from build123d import *

# Parameters (mm, degrees)
SKETCH1_R           = 5
BOSS_EXTRUDE1_DEPTH = 6
SKETCH2_R           = 3
BOSS_EXTRUDE2_DEPTH = 25
CHAMFER1_SIZE       = 0.3
CUT_EXTRUDE1_DEPTH  = 3


with BuildPart() as part:
    # Sketch1 → Boss-Extrude1 (new body)
    with BuildSketch(Plane.XY):
        Circle(SKETCH1_R)
    extrude(amount=BOSS_EXTRUDE1_DEPTH)

    # Sketch2 → Boss-Extrude2 (add)
    with BuildSketch(Plane.XY.offset(6)):
        Circle(SKETCH2_R)
    extrude(amount=BOSS_EXTRUDE2_DEPTH)

    # Chamfer1
    chamfer1_edges = [part.edges().sort_by_distance(p)[0] for p in [
        (-5, 0, 0),
        (-5, 0, 6),
    ]]
    chamfer(chamfer1_edges, length=CHAMFER1_SIZE)

    # Sketch3 → Cut-Extrude1 (cut)
    with BuildSketch(Plane(origin=(0, 0, 0), x_dir=(-1, 0, 0), z_dir=(0, 0, -1))):
        Polygon((0, 2.42932406), (-2.10385635, 1.21466203), (-2.10385635, -1.21466203), (0, -2.42932406), (2.10385635, -1.21466203), (2.10385635, 1.21466203), align=None)
    extrude(amount=-CUT_EXTRUDE1_DEPTH, mode=Mode.SUBTRACT)


solid = part.part
Can you work these out from the model? Positions are in its coordinate system, mm. A direction names the side the tool comes from. Give positions to 0.01 mm unless a question says otherwise; leave off trailing zeros. Write each loop counter-clockwise with the first axis right and the second up, starting at its lowest first coordinate (ties: lowest second). Pieces come first, ordered by that corner, then holes. Notation, with made-up numbers: (86, 29.5) -> (124, 29.5) arc R27 cw to (124, 53.5) -> close; hole circle Ø3 at (-7.75, 15.25). An arc over 180 degrees is marked (long way). Answer as a JSON object with one key per item and string values. Group by question number.
Item 1: I'm going to push flat-ended pins straight in: P1, Ø2, axis at x = 3, y = -3.5, coming from the +Z side; P2, Ø1, axis at x = 2, z = 4, coming from the -Y side; P3, Ø1.3, axis at x = -0.5, y = 1, coming from the -Z side; P4, Ø5, axis at y = 2.5, z = 5.5, coming from the +X side. Where does each tip first touch, or does it pass through?
Item 2: Suppose I cut it at A-A (y = 0). Please give me the cut outline in (x, z), plus the area to 3 significant figures.
Item 3: We'd pull the mould along Y, two halves only. Please class faces 1 (the face through (-3, 0, 18)), 2 (the face through (1, -3, 6)), 3 (the face through (-1.07, 1.81, 1.48)): +Y half, -Y half, draft (parallel to the pull), parting line (faces both ways), or undercut.
Item 4: Suppose I cut it at B-B (z = 9). Please give me the cut outline in (x, y), plus the area to 3 significant figures.
Item 5: Please list where these lines run through material, in increasing order: line 1 (Z direction, x = 2.5, y = 1.75); line 2 (X direction, y = 4, z = 2.5); line 3 (Y direction, x = -1.75, z = 2.5). Write a range as [from, to].
Item 6: For faces 4 (the face through (-1.08, -4.88, 2.96)), 5 (the face through (2.104, 0, 1)), which set-ups out of +Z, -Z, +X, -X, +Y, -Y let a thin tool reach every point of the face, with its end or its side?
Findings:
{
 "1": {"P1": "stops at z = 6", "P2": "stops at y = -4.77", "P3": "stops at z = 3", "P4": "stops at x = 5"},
 "2": {"outline": "(-5, 0.3) -> (-4.7, 0) -> (-2.1, 0) -> (-2.1, 3) -> (2.1, 3) -> (2.1, 0) -> (4.7, 0) -> (5, 0.3) -> (5, 5.7) -> (4.7, 6) -> (3, 6) -> (3, 31) -> (-3, 31) -> (-3, 6) -> (-4.7, 6) -> (-5, 5.7) -> close", "area": "197 mm²"},
 "3": {"face 1": "parting line", "face 2": "draft", "face 3": "undercut"},
 "4": {"outline": "circle Ø6 at (0, 0)", "area": "28.3 mm²"},
 "5": {"line 1": "z = [0, 6]", "line 2": "x = [-3, 3]", "line 3": "y = [-4.68, -1.42], [1.42, 4.68]"},
 "6": {"face 4": "+Z, -Z", "face 5": "-Z"}
}
